```python
from build123d import *

# Parameters (mm, degrees)
SKETCH1_R           = 5
BOSS_EXTRUDE1_DEPTH = 4


with BuildPart() as part:
    # Sketch1 → Boss-Extrude1 (new body)
    with BuildSketch(Plane.XY):
        with BuildLine():
            Line((33.433153565, 28.077762704), (17.848337966, 28.077762704))
            ThreePointArc((17.848337966, 28.077762704), (12.001235119, 26.190184555), (8.361504986, 21.240040364))
            Line((8.361504986, 21.240040364), (0.640745765, -1.922237296))
            Line((0.640745765, -1.922237296), (0.640745765, -31.922237296))
            Line((0.640745765, -31.922237296), (50.640745765, -31.922237296))
            Line((50.640745765, -31.922237296), (50.640745765, -1.922237296))
            Line((50.640745765, -1.922237296), (42.919986545, 21.240040364))
            ThreePointArc((42.919986545, 21.240040364), (39.280256412, 26.190184555), (33.433153565, 28.077762704))
        make_face()
        with Locations((25.640745765, 18.077762704)):
            Circle(SKETCH1_R, mode=Mode.SUBTRACT)
    extrude(amount=BOSS_EXTRUDE1_DEPTH)


solid = part.part
```
The listing builds one solid part. Answer for the finished solid, in the listing's coordinates (mm). Give positions to 0.01 mm unless a question says otherwise; leave off trailing zeros. Loops run counter-clockwise (first coordinate to the right, second up) from the corner with the lowest first, then second, coordinate; pieces in that order, holes last. Notation, with made-up numbers: (2, 18) - (43, 18) arc R31 cw to (43, 56) - close; hole circle Ø10 at (59, 19.25). An arc over 180 degrees is marked (long way). Answer as CSV lines item,"result". Start each with the question number.
Item 1: A cutting plane is placed at C-C on x = 47.5. Determine the outline of the cut face in (y, z).
Item 2: A cutting plane is placed at A-A on y = 19. Determine the outline of the cut face in (x, z).
Item 3: The mould has two halves that part along Y. Classify faces 1 (the face through (25, -31.922, 2)), 2 (the face through (39.35, 26.14, 1.97)), 3 (the face through (21.96, 21.46, 1.97)), 4 (the face through (0.641, -17, 2)): +Y half, -Y half, draft (parallel to the pull), parting line (faces both ways), or undercut.
Item 4: A cutting plane is placed at B-B on z = 2.45. Determine the outline of the cut face in (x, y).
Item 5: Find the intervals of material crossed by line 1 (Y direction, x = 25.5, z = 2.4); line 2 (Y direction, x = 27.5, z = 3.3); line 3 (Y direction, x = 9.5, z = 0.8), in increasing order. Write a range as from..to.
Item 6: A cutting plane is placed at D-D on x = 11.5. Determine the outline of the cut face in (y, z).
Item 7: This flat-tipped pin is pushed along its axis until it touches: pin 1 (8 mm diameter, centred on x = 11.5, y = 16, fed in from -Z). Where does it stop, or does it pass through?
Found:
1,outline,"(-31.92, 0) - (7.5, 0) - (7.5, 4) - (-31.92, 4) - close"
2,outline,"(7.61, 0) - (20.73, 0) - (20.73, 4) - (7.61, 4) - close; (30.55, 0) - (43.67, 0) - (43.67, 4) - (30.55, 4) - close"
3,face 1,"-Y half"
3,face 2,"+Y half"
3,face 3,"undercut"
3,face 4,"draft"
4,outline,"(0.64, -31.92) - (50.64, -31.92) - (50.64, -1.92) - (42.92, 21.24) arc R10 ccw to (33.43, 28.08) - (17.85, 28.08) arc R10 ccw to (8.36, 21.24) - (0.64, -1.92) - close; hole circle Ø10 at (25.64, 18.08)"
5,line 1,"y = -31.92..13.08, 23.08..28.08"
5,line 2,"y = -31.92..13.44, 22.72..28.08"
5,line 3,"y = -31.92..23.58"
6,outline,"(-31.92, 0) - (25.8, 0) - (25.8, 4) - (-31.92, 4) - close"
7,pin 1,"stops at z = 0"
